from build123d import *

# Parameters (mm, degrees)
SKETCH_1_W                = 320
SKETCH_1_H                = 80
EXTRUDE_1_DEPTH           = 12
CHAMFER_1_SIZE            = 5
HOLE_WIZARD_M8_1_D        = 6.8
HOLE_WIZARD_8_5_8_5_1_D   = 8.5
HOLE_WIZARD_1_D           = 6.6
HOLE_WIZARD_1_CBORE_D     = 11
HOLE_WIZARD_1_CBORE_DEPTH = 6.8


with BuildPart() as part:
    # 草图1 → 凸台-拉伸1 (new body)
    with BuildSketch(Plane.XY):
        Rectangle(SKETCH_1_W, SKETCH_1_H)
    extrude(amount=EXTRUDE_1_DEPTH)

    # 倒角1
    chamfer_1_edges = [part.edges().sort_by_distance(p)[0] for p in [
        (160, -40, 6),
        (-160, -40, 6),
        (-160, 40, 6),
        (160, 40, 6),
    ]]
    chamfer(chamfer_1_edges, length=CHAMFER_1_SIZE)

    # M8 螺纹孔1 (through all)
    with Locations(Plane(origin=(0, 0, 0), x_dir=(-1, 0, 0), z_dir=(0, 0, -1))):
        with Locations((-145, 9.5), (-145, -9.5), (145, 9.5), (145, -9.5)):
            Hole(HOLE_WIZARD_M8_1_D / 2)

    # Ø8.5 (8.5) 直径孔1 (through all)
    with Locations(Plane(origin=(0, 0, 0), x_dir=(-1, 0, 0), z_dir=(0, 0, -1))):
        with Locations((-145, 27.5), (-145, -27.5), (145, 27.5), (145, -27.5)):
            Hole(HOLE_WIZARD_8_5_8_5_1_D / 2)

    # 打孔尺寸(%根据)内六角圆柱头螺钉的类型1 (through all)
    with Locations(Plane.XY.offset(12)):
        with Locations((-60, 15), (0, 15), (60, 15), (100, -25), (-100, -25)):
            CounterBoreHole(HOLE_WIZARD_1_D / 2, HOLE_WIZARD_1_CBORE_D / 2, HOLE_WIZARD_1_CBORE_DEPTH)


solid = part.part
Verification items for the finished model (mm, model axes). A direction names the side the tool comes from. Round coordinates to 2 decimals unless told otherwise and drop trailing zeros. Loops run counter-clockwise (first coordinate to the right, second up) from the corner with the lowest first, then second, coordinate; pieces in that order, holes last. Notation, with made-up numbers: (-21.5, -11.75) - (7.5, -11.75) arc R12 ccw to (7.5, 8.25) - close; hole circle Ø7 at (36.5, 61.5). An arc over 180 degrees is marked (long way). Use a Markdown table: item, result. Add a question column.
1. Gauge pin test, flat end, axial feed: pin 1 (6 mm diameter, centred on x = -145, y = -9.5, fed in from -Z). Record the tip position at first contact, or that the pin passes through.
2. Section check A-A, the plane x = -145. Record the boundary of the cut face in (y, z), plus the area to 3 significant figures.
3. Section check C-C, the plane y = 27.5. Record the boundary of the cut face in (x, z), plus the area to 3 significant figures.
4. Section check D-D, the plane x = 60. Record the boundary of the cut face in (y, z), plus the area to 3 significant figures.
5. Section check B-B, the plane z = 2.25. Give the number of separate pieces and of enclosed holes in the cut face, plus the area to 3 significant figures.
6. Release check for a two-part mould opening along X. For faces 1 (the face through (-2, -40, 6)), 2 (the face through (158, -37, 6)), 3 (the face through (102.619, -27.008, 2.564)), 4 (the face through (-160, 0, 6)) record: released by +X, released by -X, zero draft, split by the parting line, or undercut.
7. Thickness scan on probe 1 along Y at (x, z) = (145, 3.5); probe 2 along X at (y, z) = (-11, 5.25); probe 3 along X at (y, z) = (16, 8). Record the ranges inside material, lowest first. Write a range as [from, to].
8. Access from +Z, -Z, +X, -X, +Y, -Y to the whole of each face (thin tool, end or side, straight path). Record for faces 5 (the face through (140.754, 27.687, 6.084)), 6 (the face through (94.505, -24.758, 8.648)).
Checks:
| question | item | result |
|---|---|---|
| 1 | pin 1 | passes through |
| 2 | outline | (-40, 0) - (-31.75, 0) - (-31.75, 12) - (-40, 12) - close; (-23.25, 0) - (-12.9, 0) - (-12.9, 12) - (-23.25, 12) - close; (-6.1, 0) - (6.1, 0) - (6.1, 12) - (-6.1, 12) - close; (12.9, 0) - (23.25, 0) - (23.25, 12) - (12.9, 12) - close; (31.75, 0) - (40, 0) - (40, 12) - (31.75, 12) - close |
| 2 | area | 593 mm^2 |
| 3 | outline | (-160, 0) - (-149.25, 0) - (-149.25, 12) - (-160, 12) - close; (-140.75, 0) - (140.75, 0) - (140.75, 12) - (-140.75, 12) - close; (149.25, 0) - (160, 0) - (160, 12) - (149.25, 12) - close |
| 3 | area | 3,640 mm^2 |
| 4 | outline | (-40, 0) - (11.7, 0) - (11.7, 5.2) - (9.5, 5.2) - (9.5, 12) - (-40, 12) - close; (18.3, 0) - (40, 0) - (40, 12) - (20.5, 12) - (20.5, 5.2) - (18.3, 5.2) - close |
| 4 | area | 851 mm^2 |
| 5 | separate pieces | 1 |
| 5 | enclosed holes | 13 |
| 5 | area | 25,000 mm^2 |
| 6 | face 1 | zero draft |
| 6 | face 2 | released by +X |
| 6 | face 3 | undercut |
| 6 | face 4 | released by -X |
| 7 | probe 1 | y = [-40, -31.75], [-23.25, -12.9], [-6.1, 6.1], [12.9, 23.25], [31.75, 40] |
| 7 | probe 2 | x = [-160, -148.05], [-141.95, 141.95], [148.05, 160] |
| 7 | probe 3 | x = [-160, -65.41], [-54.59, -5.41], [5.41, 54.59], [65.41, 160] |
| 8 | face 5 | +Z, -Z |
| 8 | face 6 | +Z |
